Geometry: final body of the model. Coordinates: model frame, mm. A direction names the side the tool comes from. Coordinates: 2 decimals unless noted, no trailing zeros. Order: outer loops, then holes, each group sorted by start corner. A loop starts at its lowest first (then second) coordinate and runs counter-clockwise, first axis right, second up. Notation, with made-up numbers: (-11.75, -19.75) - (33.25, -19.75) arc R24 ccw to (33.25, -0.75) - close; hole circle Ø7 at (68.25, -19.5). An arc over 180 degrees is marked (long way). Use one line per item in the form item = value. Start each with the question number.
```python
from build123d import *

# Parameters (mm, degrees)
EXTRUDE_1_DEPTH     = 1750
CUT_EXTRUDE_3_DEPTH = 100
CUT_REVOLVE_1_ANGLE = 90


with BuildPart() as part:
    # 草图1 → 凸台-拉伸1 (new body)
    with BuildSketch(Plane.XY):
        with BuildLine():
            Line((-130, -144.638291086), (0, -144.638291086))
            Line((0, -144.638291086), (0, -4.188946248))
            Line((0, -4.188946248), (0, 75.811053752))
            Line((0, 75.811053752), (0, 185.69710624))
            Line((0, 185.69710624), (0, 225.814837569))
            Line((0, 225.814837569), (-108.083873316, 225.814837569))
            Line((-108.083873316, 225.814837569), (-185.80387332, 225.814837569))
            Line((-185.80387332, 225.814837569), (-185.80387332, 202.814837569))
            Line((-185.80387332, 202.814837569), (-100.01423666, 173.289453092))
            add(Edge.make_bspline(
                [(-100.01423666, 173.289453092), (-89.242307137, 167.173453817), (-82.491572572, 150.19537082), (-92.192076155, 140.122990005)],
                knots=[0, 0, 0, 0, 1, 1, 1, 1], degree=3))
            Line((-92.192076155, 140.122990005), (-153.01423666, 70.814837569))
            Line((-153.01423666, 70.814837569), (-180.01423666, 70.814837569))
            Line((-180.01423666, 70.814837569), (-180.01423666, 40.814837569))
            Line((-180.01423666, 40.814837569), (-153.01423666, 40.814837569))
            Line((-153.01423666, 40.814837569), (-102.31538594, -24.896770131))
            ThreePointArc((-102.31538594, -24.896770131), (-95.998763417, -48.223878967), (-108.02699364, -69.185162431))
            Line((-108.02699364, -69.185162431), (-185.80387332, -96.42399324))
            add(Edge.make_bspline(
                [(-187.99699364, -99.18894625), (-187.738237709, -97.242367883), (-185.80387332, -96.42399324)],
                knots=[0, 0, 0, 1, 1, 1], degree=2))
            Line((-187.99699364, -99.18894625), (-187.99699364, -129.188946248))
            Line((-187.99699364, -129.188946248), (-140.299563226, -129.188946248))
            Line((-140.299563226, -129.188946248), (-130, -144.638291086))
        make_face()
    extrude(amount=-EXTRUDE_1_DEPTH)

    # 草图3 → 切除-拉伸3 (cut)
    with BuildSketch(Plane.XY):
        with BuildLine():
            Line((0, -4.638291086), (-20, -4.638291086))
            ThreePointArc((-20, -4.638291086), (-60, 35.361708914), (-20, 75.361708914))
            Line((-20, 75.361708914), (0, 75.361708914))
            Line((0, 75.361708914), (0, -4.638291086))
        make_face()
    cut_extrude_3 = extrude(amount=-CUT_EXTRUDE_3_DEPTH, mode=Mode.SUBTRACT)

    # 草图5 → 切除-旋转1 (revolve, cut)
    with BuildSketch(Plane(origin=(0, 0, 0), x_dir=(0, 0, -1), z_dir=(1, 0, 0))):
        with BuildLine():
            Line((100, 95.361708914), (100, -24.638291086))
            ThreePointArc((100, -24.638291086), (160, 35.361708914), (100, 95.361708914))
        make_face()
    cut_revolve_1 = revolve(axis=Axis((0, 95.361708914, -100), (0, 1, 0)), revolution_arc=CUT_REVOLVE_1_ANGLE, mode=Mode.SUBTRACT)

    # 镜向1: 切除-拉伸3, 切除-旋转1 across plane
    add(cut_extrude_3.mirror(Plane.XY.offset(-875)), mode=Mode.SUBTRACT)
    add(cut_revolve_1.mirror(Plane.XY.offset(-875)), mode=Mode.SUBTRACT)


solid = part.part
```
(1) Set-up query: faces 1 (the cylindrical face through (-59.99, 34.48, -49.3)), 2 (the flat face through (-166, 70.815, -863)), 3 (the flat face through (-164, -129.189, -863)). Return all of +Z, -Z, +X, -X, +Y, -Y with unobstructed straight access to the full face (end or side cutting, diameter ignored); none if empty.
(2) Draft query along Z for faces 4 (the flat face through (-23, 79, -100)), 5 (the flat face through (-74, 43, 0)), 6 (the flat face through (-92, 225.815, -863)). Return one class per face: released by +Z, released by -Z, zero draft, split by the parting line, or undercut.
(3) Cut plane A-A on x = -40. Return the cut outline in (y, z), plus the area to 3 significant figures.
(4) Material intervals for L1, parallel to Y at x = -156, z = -1046.5; L2, parallel to Z at x = -17, y = -14; L3, parallel to Y at x = -166, z = -1129, sorted ascending. Write a range as from..to.
(5) Contact query for flat-ended pins moving along their axis: pin 1 Ø7 at (y, z) = (213, -609) entering from -X; pin 2 Ø15 at (y, z) = (59, -1030) entering from -X. Output: stop coordinate, or through.
Check sheet entries:
q1.face_1 = +Z, +X
q1.face_2 = +Z, -Z, -X
q1.face_3 = +Z, -Z, -X, -Y
q2.face_4 = undercut
q2.face_5 = released by +Z
q2.face_6 = zero draft
q3.outline = (-144.64, -1750) - (0.72, -1750) - (0.72, -1650) - (-9.36, -1650) arc R44.72 cw to (80.08, -1650) - (70, -1650) - (70, -1750) - (225.81, -1750) - (225.81, 0) - (70, 0) - (70, -100) - (80.08, -100) arc R44.72 cw to (-9.36, -100) - (0.72, -100) - (0.72, 0) - (-144.64, 0) - close
q3.area = 628,000 mm^2
q4.L1 = -129.19..-85.99, 40.81..70.81, 192.56..225.81
q4.L2 = -1750..-1650, -1620.43..-129.57, -100..0
q4.L3 = -129.19..-89.49, 40.81..70.81, 196..225.81
q5.pin_1 = -185.8
q5.pin_2 = -180.01
